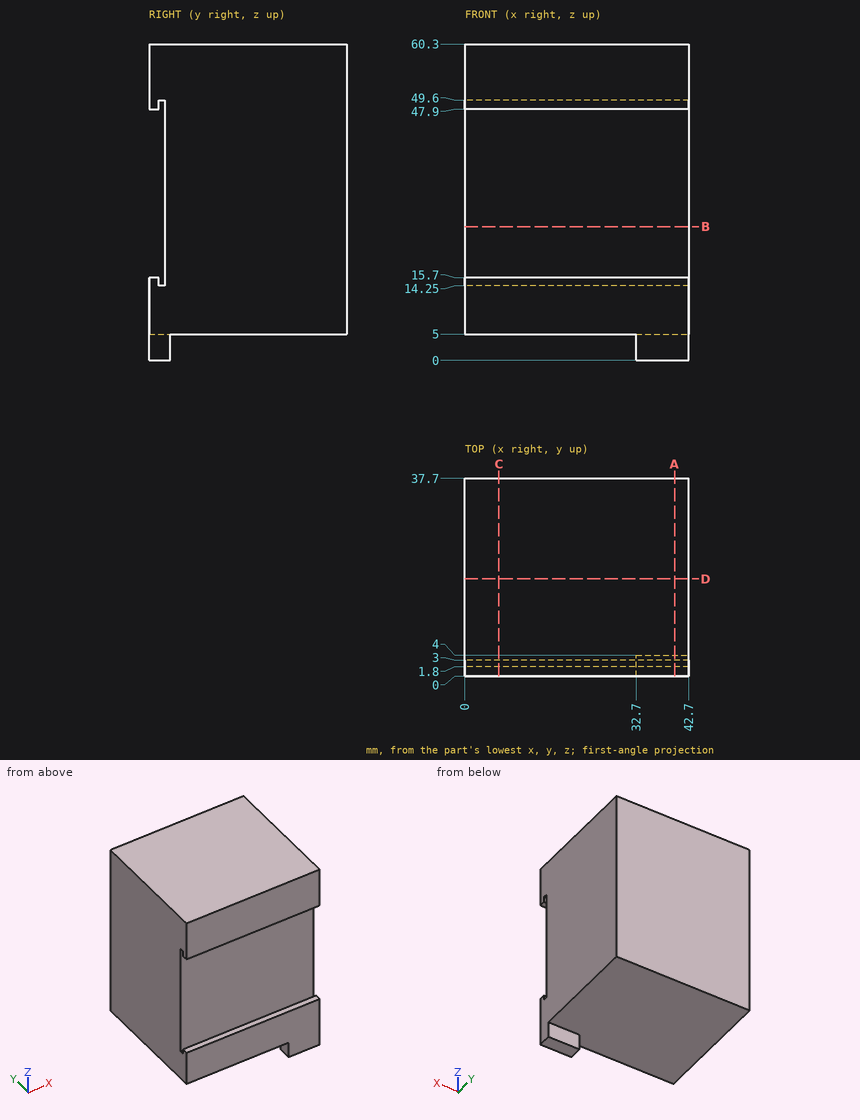
Verification items for this drawing (mm, ordinates from the low corner). Coordinates: 2 decimals unless noted, no trailing zeros. Write each loop counter-clockwise with the first axis right and the second up, starting at its lowest first coordinate (ties: lowest second). Pieces come first, ordered by that corner, then holes. Notation, with made-up numbers: M 11,35.5 L 26,35.5 A14 cw 26,52.5 Z; hole C 45.5,59 d9. An arc over 180 degrees is marked long. Use CSV: the item, a comma, the result in double quotes.
Q1. Section check C-C, the plane x = 6.5. Enter the section's corners in (y, z).
Computed values:
outline,"M 0,5 L 37.7,5 L 37.7,60.3 L 0,60.3 L 0,47.9 L 1.8,47.9 L 1.8,49.6 L 3,49.6 L 3,14.25 L 1.8,14.25 L 1.8,15.7 L 0,15.7 Z"
Q2. Thickness scan on line 1 along Z through (x, y) = (21, 21); line 2 along Y through (x, z) = (32, 21); line 3 along Y through (x, z) = (6.5, 14.5). Record the ranges inside material, lowest first. Write a range as [from, to].
Computed values:
line 1,"[5, 60.3]"
line 2,"[3, 37.7]"
line 3,"[0, 1.8], [3, 37.7]"
Q3. Section check D-D, the plane y = 18.5. Enter the section's corners in (x, z).
Computed values:
outline,"M 0,5 L 42.7,5 L 42.7,60.3 L 0,60.3 Z"
Q4. Section check A-A, the plane x = 40. Enter the section's corners in (y, z).
Computed values:
outline,"M 0,0 L 4,0 L 4,5 L 37.7,5 L 37.7,60.3 L 0,60.3 L 0,47.9 L 1.8,47.9 L 1.8,49.6 L 3,49.6 L 3,14.25 L 1.8,14.25 L 1.8,15.7 L 0,15.7 Z"
Q5. Go/stop test with flat-tipped pins: P1, Ø0.9, axis at x = 12, y = 1, coming from the -Z side; P2, Ø6, axis at x = 16, z = 8.5, coming from the -Y side; P3, Ø3, axis at x = 22.5, z = 40, coming from the -Y side; P4, Ø4, axis at x = 35.5, z = 2, coming from the +Y side. Record where each tip stops, or that it passes through.
Computed values:
P1,"z = 5"
P2,"y = 0"
P3,"y = 3"
P4,"y = 4"
Q6. Section check B-B, the plane z = 25.5. Enter the section's corners in (x, y).
Computed values:
outline,"M 0,3 L 42.7,3 L 42.7,37.7 L 0,37.7 Z"
